from build123d import *

# Parameters (mm, degrees)
SKETCH_1_R          = 3
EXTRUDE_1_DEPTH     = 7.5
HOLE_WIZARD_M4_1_D  = 3.3
SKETCH_5_R          = 2.25
CUT_EXTRUDE_1_DEPTH = 10
CHAMFER_1_SIZE      = 1


with BuildPart() as part:
    # 草图1 → 凸台-拉伸1 (new, symmetric)
    with BuildSketch(Plane(origin=(0, 0, 0), x_dir=(1, 0, 0), z_dir=(0, 1, 0))):
        with BuildLine():
            Line((-8, 0), (-8, 29))
            Line((-8, 29), (-16.5, 29))
            Line((-16.5, 29), (-16.5, 37))
            Line((-16.5, 37), (16.5, 37))
            Line((16.5, 37), (16.5, 29))
            Line((16.5, 29), (8, 29))
            Line((8, 29), (8, 0))
            ThreePointArc((8, 0), (0, -8), (-8, 0))
        make_face()
        with Locations(Location((0, 0, 0), (0, 0, 270))):
            Circle(SKETCH_1_R, mode=Mode.SUBTRACT)
    extrude(amount=EXTRUDE_1_DEPTH, both=True)

    # M4 螺纹孔1 (through all)
    with Locations(Plane(origin=(8, 0, 0), x_dir=(0, 0, -1), z_dir=(1, 0, 0))):
        with Locations((2, 0)):
            Hole(HOLE_WIZARD_M4_1_D / 2)

    # 草图5 → 切除-拉伸1 (cut)
    with BuildSketch(Plane.XY.offset(-29)):
        with Locations((-12.5, 0)):
            Circle(SKETCH_5_R)
        with Locations((12.5, 0)):
            Circle(SKETCH_5_R)
    extrude(amount=-CUT_EXTRUDE_1_DEPTH, mode=Mode.SUBTRACT)

    # 倒角1
    chamfer_1_edges = [part.edges().sort_by_distance(p)[0] for p in [
        (16.5, 7.5, -33),
        (-16.5, 7.5, -33),
        (-16.5, -7.5, -33),
        (16.5, -7.5, -33),
    ]]
    chamfer(chamfer_1_edges, length=CHAMFER_1_SIZE)


solid = part.part
The model under review builds one solid part; all positions refer to its coordinate system, in mm. A direction names the side the tool comes from. Round coordinates to 2 decimals unless told otherwise and drop trailing zeros. Loops run counter-clockwise (first coordinate to the right, second up) from the corner with the lowest first, then second, coordinate; pieces in that order, holes last. Notation, with made-up numbers: M 64.25,4 L 69.25,4 A19 cw 69.25,16 Z; hole C 74,80 d2. An arc over 180 degrees is marked long. Answer as a JSON object with one key per item and string values.
Item 1: The part is to be moulded in two halves that separate along X. For faces 1 (the face through (-14.748, 0.099, -32.944)), 2 (the face through (16, 7, -33)), 3 (the face through (0, 0, -37)), say which applies: +X half, -X half, draft (parallel to the pull), parting line (faces both ways), or undercut.
Check sheet entries:
{"face 1": "undercut", "face 2": "+X half", "face 3": "draft"}
Item 2: We need section B-B, the plane y = 3.25. State the section outline as (x, z) points.
Check sheet entries:
{"outline": "M -16.5,-37 L 16.5,-37 L 16.5,-29 L 8,-29 L 8,0 A8 ccw -8,0 L -8,-29 L -16.5,-29 Z; hole C 0,0 d6"}
Item 3: For line 1 along Y through (x, z) = (-12.5, -31.5); line 2 along Z through (x, y) = (0, -1.75); line 3 along Y through (x, z) = (4.5, -2.5), list the stretches that pass through material, from the lowest coordinate up.
Check sheet entries:
{"line 1": "-7.5 to -2.25, 2.25 to 7.5", "line 2": "-37 to -3, 3 to 8", "line 3": "-7.5 to -1.57, 1.57 to 7.5"}
Item 4: We need section C-C, the plane z = -2. State the section outline as (x, y) points, and give its area (3 significant figures).
Check sheet entries:
{"outline": "M -8,-7.5 L -2.24,-7.5 L -2.24,-1.65 L -8,-1.65 Z; M -8,1.65 L -2.24,1.65 L -2.24,7.5 L -8,7.5 Z; M 2.24,-7.5 L 8,-7.5 L 8,-1.65 L 2.24,-1.65 Z; M 2.24,1.65 L 8,1.65 L 8,7.5 L 2.24,7.5 Z", "area": "135 mm2"}
Item 5: Tool access review of faces 4 (the face through (16.5, 0, -33)), 5 (the face through (-10, 2, -29)), 6 (the face through (14, 2, -29)): name each direction out of +Z, -Z, +X, -X, +Y, -Y from which nothing blocks a thin tool from reaching the whole face with its end or side.
Check sheet entries:
{"face 4": "+Z, -Z, +X, +Y, -Y", "face 5": "+Z, -X, +Y, -Y", "face 6": "+Z, +X, +Y, -Y"}
Item 6: We need section D-D, the plane y = 0. State the section outline as (x, z) points, and give its area (4 significant figures).
Check sheet entries:
{"outline": "M -16.5,-37 L -14.75,-37 L -14.75,-29 L -16.5,-29 Z; M -10.25,-37 L 10.25,-37 L 10.25,-29 L 8,-29 L 8,-3.65 L -8,-3.65 L -8,-29 L -10.25,-29 Z; M -8,-0.35 L -2.98,-0.35 A3 cw long 2.98,-0.35 L 8,-0.35 L 8,0 A8 ccw -8,0 Z; M 14.75,-37 L 16.5,-37 L 16.5,-29 L 14.75,-29 Z", "area": "687.5 mm2"}
Item 7: Clearance check with flat-ended pins moving along their axes: P1, Ø8, axis at y = -1, z = -12, coming from the +X side; P2, Ø3, axis at x = -2.5, y = -4, coming from the +Z side; P3, Ø7, axis at x = 12.5, y = -1, coming from the +Z side. State where each tip first meets the part, or that it passes through.
Check sheet entries:
{"P1": "x = 8", "P2": "z = 7.94", "P3": "z = -29"}
Item 8: We need section A-A, the plane x = 12.5. State the section outline as (y, z) points.
Check sheet entries:
{"outline": "M -7.5,-37 L -2.25,-37 L -2.25,-29 L -7.5,-29 Z; M 2.25,-37 L 7.5,-37 L 7.5,-29 L 2.25,-29 Z"}
